from build123d import *

# Parameters (mm, degrees)
SKETCH_1_W                = 10
SKETCH_1_H                = 225
EXTRUDE_1_DEPTH           = 12.5
CHAMFER_1_SIZE            = 20
CHAMFER_1_SIZE2           = 5.358983849
HOLE_WIZARD_1_D           = 4.8
HOLE_WIZARD_1_CBORE_D     = 8
HOLE_WIZARD_1_CBORE_DEPTH = 5
HOLE_WIZARD_M4_1_D        = 3.3
FILLET_1_R                = 10


with BuildPart() as part:
    # 草图1 → 凸台-拉伸1 (new, symmetric)
    with BuildSketch(Plane(origin=(0, 0, 0), x_dir=(0, 0, -1), z_dir=(1, 0, 0))):
        Rectangle(SKETCH_1_W, SKETCH_1_H)
    extrude(amount=EXTRUDE_1_DEPTH, both=True)

    # 倒角1
    chamfer_1_edges = [part.edges().sort_by_distance(p)[0] for p in [
        (0, 112.5, -5),
    ]]
    chamfer_1_side = [part.faces().sort_by_distance(p)[0] for p in [
        (0, 0, -5),
    ]]
    chamfer(chamfer_1_edges, length=CHAMFER_1_SIZE, length2=CHAMFER_1_SIZE2, reference=chamfer_1_side[0])

    # 打孔尺寸(%根据)开槽圆柱头螺钉的类型1 (through all)
    with Locations(Plane.ZY.offset(12.5)):
        with Locations((0, 75), (0, 0), (0, -75)):
            CounterBoreHole(HOLE_WIZARD_1_D / 2, HOLE_WIZARD_1_CBORE_D / 2, HOLE_WIZARD_1_CBORE_DEPTH)

    # M4 螺纹孔1 (through all)
    with Locations(Plane.XY.offset(5)):
        with Locations((0, 45), (0, -35)):
            Hole(HOLE_WIZARD_M4_1_D / 2)

    # 圆角1
    fillet_1_edges = [part.edges().sort_by_distance(p)[0] for p in [
        (0, 92.5, -5),
    ]]
    fillet(fillet_1_edges, radius=FILLET_1_R)


solid = part.part
Source: CAD feature listing. Evaluate the final solid. Frame: model axes, mm. A direction names the side the tool comes from. Round coordinates to 2 decimals unless told otherwise and drop trailing zeros. Loops run counter-clockwise (first coordinate to the right, second up) from the corner with the lowest first, then second, coordinate; pieces in that order, holes last. Notation, with made-up numbers: M 35.5,67 L 68.5,67 A17 cw 68.5,99 Z; hole C 48.5,-24.75 d6. An arc over 180 degrees is marked long. Return JSON: item names as keys, results as strings. Group by question number.
1. Reachability of faces 1 (the face through (-7.5, -77, 2)), 2 (the face through (2.64, -72.62, 0.31)) from +Z, -Z, +X, -X, +Y, -Y: full face, straight path, thin tool, end or side. Return the list, or none.
2. Section query A-A on y = -75. Output: boundary loops of the cut face in (x, z), and give its area (3 significant figures).
3. Section query B-B on x = 6.25. Output: boundary loops of the cut face in (y, z).
4. Pin query (flat end, axial travel): pin 1 (2.5 mm diameter, centred on y = -76, z = 1.5, fed in from -X). Return the tip coordinate at first contact, or that it passes through.
5. Material intervals for line 1 along Y through (x, z) = (0, 3); line 2 along Y through (x, z) = (10.25, 1.75), sorted ascending. Write a range as from..to.
6. Mould query, pull axis Z, two halves, no side actions, for faces 3 (the face through (2.64, 77.38, 0.31)), 4 (the face through (0, -112.5, 0)), 5 (the face through (0, -2, 5)). Classes: released by +Z, released by -Z, zero draft, split by the parting line, or undercut.
Checks:
{
 "1": {"face 1": "-X", "face 2": "+X, -X"},
 "2": {"outline": "M -12.5,-5 L 12.5,-5 L 12.5,-2.4 L -7.5,-2.4 L -7.5,-4 L -12.5,-4 Z; M -12.5,4 L -7.5,4 L -7.5,2.4 L 12.5,2.4 L 12.5,5 L -12.5,5 Z", "area": "114 mm²"},
 "3": {"outline": "M -112.5,-5 L 91.18,-5 A10 ccw 93.77,-4.66 L 112.5,0.36 L 112.5,5 L -112.5,5 Z; hole C -75,0 d4.8; hole C 0,0 d4.8; hole C 75,0 d4.8"},
 "4": {"pin 1": "stops at x = -7.5"},
 "5": {"line 1": "y = -112.5..-36.65, -33.35..43.35, 46.65..112.5", "line 2": "y = -112.5..-76.64, -73.36..-1.64, 1.64..73.36, 76.64..112.5"},
 "6": {"face 3": "undercut", "face 4": "zero draft", "face 5": "released by +Z"}
}
